from build123d import *

# Parameters (mm, degrees)
BOSS_EXTRUDE1_DEPTH = 1.5


with BuildPart() as part:
    # Sketch1 → Boss-Extrude1 (new body)
    with BuildSketch(Plane.XY):
        Polygon((-17.5, 17.5), (22.5, -12.5), (22.5, -17.5), (-20.5, -17.5), (-22.5, -15.5), (-22.5, 17.5), align=None)
    extrude(amount=BOSS_EXTRUDE1_DEPTH)


solid = part.part
Geometry: final body of the model. Coordinates: model frame, mm. Give positions to 0.01 mm unless a question says otherwise; leave off trailing zeros. Loops run counter-clockwise (first coordinate to the right, second up) from the corner with the lowest first, then second, coordinate; pieces in that order, holes last. Notation, with made-up numbers: (51.5, 79.5) - (81.5, 79.5) arc R36 ccw to (81.5, 116.5) - close; hole circle Ø11 at (6.5, 23). An arc over 180 degrees is marked (long way). One line per question, with ' | ' between items. Start each with the question number.
(1) Section query A-A on y = 1. Return loops of the section in (x, z).
(2) Section query C-C on x = 11. Return loops of the section in (y, z) (3 decimals), then the cut area to 3 significant figures.
(3) Section query B-B on z = 1.25. Return loops of the section in (x, y), then the cut area to 3 significant figures.
(4) Ray query, line 1 (Y direction, x = 5.5, z = 1.3); line 2 (Y direction, x = -7, z = 1.2) (3 decimals); line 3 (X direction, y = 0, z = 0.2). Return the intervals inside material, ascending. Write a range as from..to.
The answers:
1) outline: (-22.5, 0) - (4.5, 0) - (4.5, 1.5) - (-22.5, 1.5) - close
2) outline: (-17.5, 0) - (-3.875, 0) - (-3.875, 1.5) - (-17.5, 1.5) - close | area: 20.4 mm2
3) outline: (-22.5, -15.5) - (-20.5, -17.5) - (22.5, -17.5) - (22.5, -12.5) - (-17.5, 17.5) - (-22.5, 17.5) - close | area: 973 mm2
4) line 1: -17.5..0.25 | line 2: -17.5..9.625 | line 3: -22.5..5.83
